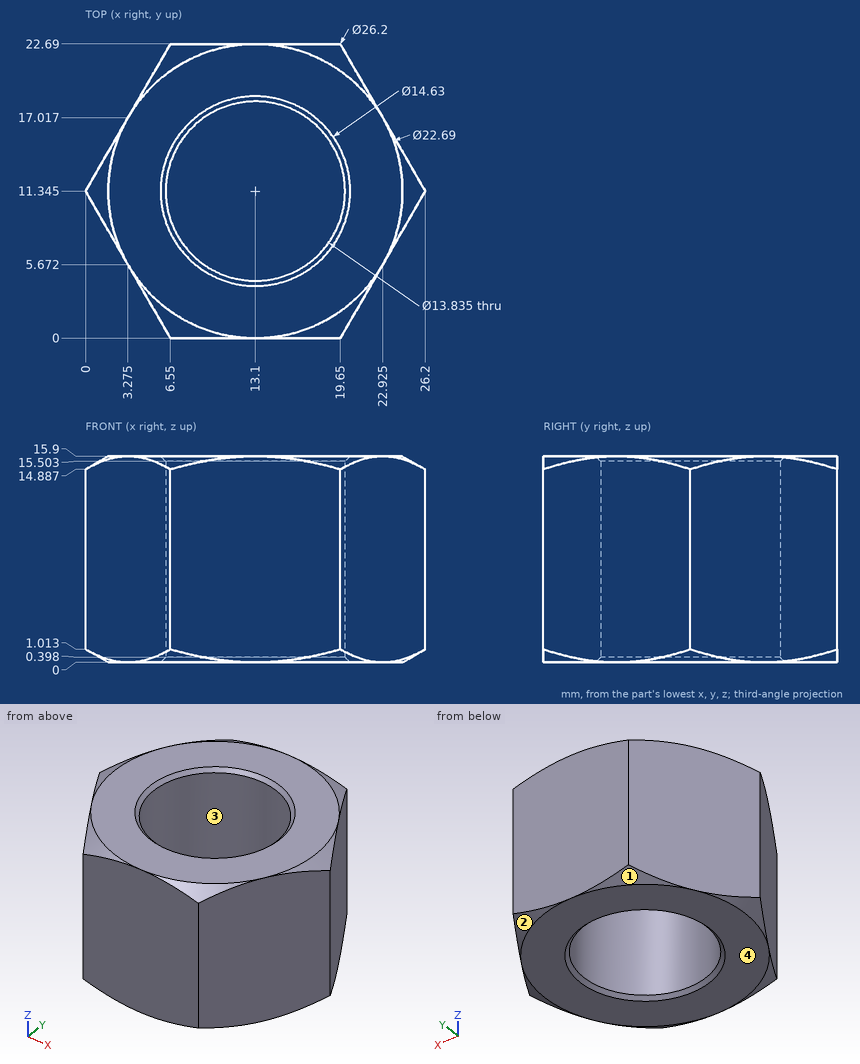
Drawing for the job (mm, zero at the part's lowest x, y, z). Give positions to 0.01 mm unless a question says otherwise; leave off trailing zeros.
(1) Drill centre lines: line 1 along X through (y, z) = (16.5, 8.75) (1 decimal); line 2 along X through (y, z) = (16.25, 2) (1 decimal); line 3 along X through (y, z) = (1.75, 10). Where is each one in solid material? Low to high.
Return value:
line 1: x = 3 to 8.5, 17.7 to 23.2
line 2: x = 2.8 to 8.2, 18 to 23.4
line 3: x = 5.54 to 20.66
(2) Pull direction X, two halves, no side cores. Call the marked faces 1, 2, 3 and 4: pulls with the +X half, pulls with the -X half, needs draft (parallel to the pull), parting line crosses it, or undercut.
Return value:
face 1: pulls with the -X half
face 2: pulls with the +X half
face 3: undercut
face 4: needs draft
(3) Pin check, flat tips, straight feed: pin 1 (2 mm diameter, centred on y = 19, z = 13.5, fed in from -X); pin 2 (6 mm diameter, centred on y = 7.5, z = 9, fed in from -X); pin 3 (4 mm diameter, centred on x = 23, z = 11.5, fed in from +Y). Stop position of each tip, or through.
Return value:
pin 1: stops at x = 3.84
pin 2: stops at x = 0.49
pin 3: stops at y = 20.35
